```python
from build123d import *

# Parameters (mm, degrees)
SKETCH1_W              = 300
SKETCH1_H              = 220
BOSS_EXTRUDE1_DEPTH    = 10
SKETCH3_R              = 66
CUT_EXTRUDE1_DEPTH     = 187.279360102
M10_TAPPED_HOLE1_D     = 8.5
M10_TAPPED_HOLE1_DEPTH = 24.5
M10_TAPPED_HOLE1_TIP   = 2.553657631
CUT_EXTRUDE2_DEPTH     = 187.279360102
FILLET1_R              = 5


with BuildPart() as part:
    # Sketch1 → Boss-Extrude1 (new body)
    with BuildSketch(Plane(origin=(0, 0, 0), x_dir=(1, 0, 0), z_dir=(0, 1, 0))):
        Rectangle(SKETCH1_W, SKETCH1_H)
    extrude(amount=BOSS_EXTRUDE1_DEPTH)

    # Sketch3 → Cut-Extrude1 (cut, through all)
    with BuildSketch(Plane(origin=(0, 10, 0), x_dir=(1, 0, 0), z_dir=(0, 1, 0))):
        with Locations(Location((0, 0, 0), (0, 0, 270))):
            Circle(SKETCH3_R)
    extrude(amount=-CUT_EXTRUDE1_DEPTH, mode=Mode.SUBTRACT)

    # M10 Tapped Hole1
    with Locations(Plane(origin=(0, 10, 0), x_dir=(1, 0, 0), z_dir=(0, 1, 0))):
        with Locations((-58.336309448, -58.336309448), (-58.336309448, 58.336309448), (58.336309448, 58.336309448), (58.336309448, -58.336309448)):
            Hole(M10_TAPPED_HOLE1_D / 2, depth=M10_TAPPED_HOLE1_DEPTH)
            with Locations((0, 0, -(M10_TAPPED_HOLE1_DEPTH + M10_TAPPED_HOLE1_TIP / 2))):  # 118° drill point
                Cone(0, M10_TAPPED_HOLE1_D / 2, M10_TAPPED_HOLE1_TIP, mode=Mode.SUBTRACT)

    # Sketch6 → Cut-Extrude2 (cut, through all)
    with BuildSketch(Plane(origin=(0, 10, 0), x_dir=(1, 0, 0), z_dir=(0, 1, 0))):
        with BuildLine():
            Line((-135, 95.5), (-125, 95.5))
            ThreePointArc((-125, 95.5), (-119.5, 90), (-125, 84.5))
            Line((-125, 84.5), (-135, 84.5))
            ThreePointArc((-135, 84.5), (-140.5, 90), (-135, 95.5))
        make_face()
        with BuildLine():
            Line((135, 95.5), (125, 95.5))
            ThreePointArc((125, 95.5), (119.5, 90), (125, 84.5))
            Line((125, 84.5), (135, 84.5))
            ThreePointArc((135, 84.5), (140.5, 90), (135, 95.5))
        make_face()
        with BuildLine():
            Line((135, -95.5), (125, -95.5))
            ThreePointArc((125, -95.5), (119.5, -90), (125, -84.5))
            Line((125, -84.5), (135, -84.5))
            ThreePointArc((135, -84.5), (140.5, -90), (135, -95.5))
        make_face()
        with BuildLine():
            Line((-135, -95.5), (-125, -95.5))
            ThreePointArc((-125, -95.5), (-119.5, -90), (-125, -84.5))
            Line((-125, -84.5), (-135, -84.5))
            ThreePointArc((-135, -84.5), (-140.5, -90), (-135, -95.5))
        make_face()
    extrude(amount=-CUT_EXTRUDE2_DEPTH, mode=Mode.SUBTRACT)

    # Fillet1
    fillet1_edges = [part.edges().sort_by_distance(p)[0] for p in [
        (150, 5, 110),
        (-150, 5, 110),
        (-150, 5, -110),
        (150, 5, -110),
    ]]
    fillet(fillet1_edges, radius=FILLET1_R)


solid = part.part
```
Input: part model. Units: mm. Frame: model coordinates. A direction names the side the tool comes from. Coordinates: 2 decimals unless noted, no trailing zeros. Loops run counter-clockwise (first coordinate to the right, second up) from the corner with the lowest first, then second, coordinate; pieces in that order, holes last. Notation, with made-up numbers: M -36,-27.75 L -1,-27.75 A14 ccw -1,-15.75 Z; hole C 41,30 d7. An arc over 180 degrees is marked long. Use a Markdown table: item, result. Add a question column.
1) Set-up query: faces 1 (the cylindrical face through (-119.5, 5.1, -90.1)), 2 (the flat face through (-2, 5, 110)). Return all of +Z, -Z, +X, -X, +Y, -Y with unobstructed straight access to the full face (end or side cutting, diameter ignored); none if empty.
2) Section C-C, the plane x = 131. Return the cut outline in (y, z).
3) Draft query along X for faces 3 (the flat face through (150, 5, 1)), 4 (the flat face through (-130, 5, -84.5)), 5 (the flat face through (-150, 5, 1)), 6 (the flat face through (-69, 0, -2)). Return one class per face: +X half, -X half, draft (parallel to the pull), parting line (faces both ways), or undercut.
4) Section A-A, the plane x = 0. Return the cut outline in (y, z).
5) Line query: L1, parallel to Z at x = 134, y = 2.5; L2, parallel to X at y = 3.25, z = -85; L3, parallel to X at y = 4.25, z = 25. Output: solid intervals per line, ascending. Write a range as from..to.
6) Section D-D, the plane z = 0. Return the cut outline in (x, y).
7) Section B-B, the plane z = -90. Return the cut outline in (x, y).
Answer below:
| question | item | result |
|---|---|---|
| 1 | face 1 | +Y, -Y |
| 1 | face 2 | +Z, +X, -X, +Y, -Y |
| 2 | outline | M 0,-110 L 10,-110 L 10,-95.5 L 0,-95.5 Z; M 0,-84.5 L 10,-84.5 L 10,84.5 L 0,84.5 Z; M 0,95.5 L 10,95.5 L 10,110 L 0,110 Z |
| 3 | face 3 | +X half |
| 3 | face 4 | undercut |
| 3 | face 5 | -X half |
| 3 | face 6 | draft |
| 4 | outline | M 0,-110 L 10,-110 L 10,-66 L 0,-66 Z; M 0,66 L 10,66 L 10,110 L 0,110 Z |
| 5 | L1 | -110..-95.5, -84.5..84.5, 95.5..110 |
| 5 | L2 | -150..-137.29, -122.71..122.71, 137.29..150 |
| 5 | L3 | -150..-61.08, 61.08..150 |
| 6 | outline | M -150,0 L -66,0 L -66,10 L -150,10 Z; M 66,0 L 150,0 L 150,10 L 66,10 Z |
| 7 | outline | M -150,0 L -140.5,0 L -140.5,10 L -150,10 Z; M -119.5,0 L 119.5,0 L 119.5,10 L -119.5,10 Z; M 140.5,0 L 150,0 L 150,10 L 140.5,10 Z |
